```python
from build123d import *

# Parameters (mm, degrees)
BASE_PLATE_SKETCH_W        = 120
BASE_PLATE_SKETCH_H        = 72
BASE_PLATE_120X72X18_DEPTH = 9
CLAMP_RING_SKETCH_R        = 30
CLAMP_RING_SKETCH_R_2      = 24
CLAMP_RING_DEPTH           = 22
ARM_REACH                  = 190.308
ARM_END_RADIUS             = 30
ARM_PROFILE_SKETCH_W       = 26
ARM_PROFILE_SKETCH_H       = 48
CLAMP_LUG_DEPTH            = 13
CLAMP_LUG_EXTENSION_DEPTH  = 58
CLAMP_BOLT_HOLE_SKETCH_R   = 6
CLAMP_BOLT_HOLE_12_DEPTH   = 78
CLAMP_SPLIT_SLOT_SKETCH_W  = 44
CLAMP_SPLIT_SLOT_SKETCH_H  = 4
CLAMP_SPLIT_SLOT_4MM_DEPTH = 78
MOUNTING_SLOTS_2X_DEPTH    = 78


with BuildPart() as part:
    # Base Plate Sketch → Base Plate 120x72x18 (new, symmetric)
    with BuildSketch(Plane.XY):
        with Locations((60, 36)):
            Rectangle(BASE_PLATE_SKETCH_W, BASE_PLATE_SKETCH_H)
    extrude(amount=BASE_PLATE_120X72X18_DEPTH, both=True)



with BuildPart() as body_2:
    # Clamp Ring Sketch → Clamp Ring (new, symmetric)
    with BuildSketch(Plane(origin=(60, 0, 0), x_dir=(0, 0, -1), z_dir=(1, 0, 0))):
        with Locations(Location((-105, 36, 0), (0, 0, 180))):
            Circle(CLAMP_RING_SKETCH_R)
        with Locations(Location((-105, 36, 0), (0, 0, 180))):
            Circle(CLAMP_RING_SKETCH_R_2, mode=Mode.SUBTRACT)
    extrude(amount=CLAMP_RING_DEPTH, both=True)


with BuildPart() as part_1:
    add(part.part)

    add(body_2.part)  # Arm merges body 2
    # Arm: up to this cylinder (the profile starts outside it)
    arm_end = Plane(origin=(60, 36, 105), z_dir=(-1, 0, 0)) * Cylinder(ARM_END_RADIUS, 441.616, mode=Mode.PRIVATE)
    # Arm Profile Sketch → Arm (add, up to the surface)
    with BuildSketch(Plane.XY.offset(9), mode=Mode.PRIVATE) as arm_sk1:
        with Locations((60, 36)):
            Rectangle(ARM_PROFILE_SKETCH_W, ARM_PROFILE_SKETCH_H)
    arm_tool1 = extrude(arm_sk1.sketch, amount=ARM_REACH, mode=Mode.PRIVATE) - arm_end
    add(arm_tool1.solids().sort_by_distance((60, 36, 9))[0])

    # Clamp Lug Sketch → Clamp Lug (add, symmetric)
    with BuildSketch(Plane(origin=(60, 0, 0), x_dir=(0, 0, -1), z_dir=(1, 0, 0))):
        with BuildLine():
            Line((-153, 7), (-153, 65))
            Line((-153, 65), (-112.681145748, 65))
            ThreePointArc((-112.681145748, 65), (-135, 36), (-112.681145748, 7))
            Line((-112.681145748, 7), (-153, 7))
        make_face()
    extrude(amount=CLAMP_LUG_DEPTH, both=True)

    # Clamp Lug Extension Sketch → Clamp Lug Extension (add)
    with BuildSketch(Plane.XZ.offset(-7)):
        with BuildLine():
            Line((47, 153), (73, 153))
            ThreePointArc((73, 153), (60, 166), (47, 153))
        make_face()
    extrude(amount=-CLAMP_LUG_EXTENSION_DEPTH)

    # Clamp Bolt Hole Sketch → Clamp Bolt Hole Ø12 (cut)
    with BuildSketch(Plane.XZ.offset(-7)):
        with Locations(Location((60, 153, 0), (0, 0, 270))):
            Circle(CLAMP_BOLT_HOLE_SKETCH_R)
    extrude(amount=-CLAMP_BOLT_HOLE_12_DEPTH, mode=Mode.SUBTRACT)

    # Clamp Split Slot Sketch → Clamp Split Slot 4mm (cut)
    with BuildSketch(Plane.XY.offset(166)):
        with Locations((60, 35.211886187)):
            Rectangle(CLAMP_SPLIT_SLOT_SKETCH_W, CLAMP_SPLIT_SLOT_SKETCH_H)
    extrude(amount=-CLAMP_SPLIT_SLOT_4MM_DEPTH, mode=Mode.SUBTRACT)

    # Mounting Slots Sketch → Mounting Slots 2x (cut)
    with BuildSketch(Plane.XY.offset(9)):
        with BuildLine():
            Line((20.132428188, 47), (20.132428188, 25))
            ThreePointArc((20.132428188, 25), (14.132428188, 19), (8.132428188, 25))
            Line((8.132428188, 25), (8.132428188, 47))
            ThreePointArc((8.132428188, 47), (14.132428188, 53), (20.132428188, 47))
        make_face()
        with BuildLine():
            Line((99.867571812, 47), (99.867571812, 25))
            ThreePointArc((99.867571812, 25), (105.867571812, 19), (111.867571812, 25))
            Line((111.867571812, 25), (111.867571812, 47))
            ThreePointArc((111.867571812, 47), (105.867571812, 53), (99.867571812, 47))
        make_face()
    extrude(amount=-MOUNTING_SLOTS_2X_DEPTH, mode=Mode.SUBTRACT)


solid = part_1.part
```
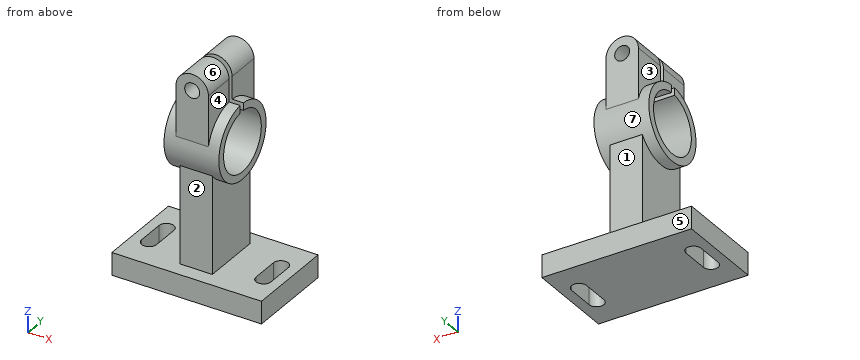
Geometry check sheet. Reference: the model listing, model coordinates, mm. Face numbers are marked on the shaded views. A direction names the side the tool comes from. Give positions to 0.01 mm unless a question says otherwise; leave off trailing zeros. Write each loop counter-clockwise with the first axis right and the second up, starting at its lowest first coordinate (ties: lowest second). Pieces come first, ordered by that corner, then holes.
1) Section check D-D, the plane y = 42.5. State how many separate pieces and enclosed holes the cut face has, and give its area (3 significant figures).
2) Release check for a two-part mould opening along Z. For the marked faces 5, 6 and 7 record: pulls with the +Z half, pulls with the -Z half, needs draft (parallel to the pull), parting line crosses it, or undercut.
3) Section check A-A, the plane z = 105. Record the boundary of the cut face in (x, y).
4) Access from +Z, -Z, +X, -X, +Y, -Y to the whole of each face (thin tool, end or side, straight path). Record for the marked faces 1, 2, 3 and 4.
5) Gauge pin test, flat ends, axial feed: pin 1 (8 mm diameter, centred on y = 24, z = 137.5, fed in from +X); pin 2 (13 mm diameter, centred on x = 64, z = 126.5, fed in from -Y); pin 3 (21 mm diameter, centred on x = 63, z = 148.5, fed in from +Y). Record the tip position at first contact, or that the pin passes through.
6) Section check C-C, the plane x = 16.5. Record the boundary of the cut face in (y, z).
7) Section check B-B, the plane y = 14. Record the boundary of the cut face in (x, z).
8) Material ranges on L1, parallel to X at y = 27.5, z = 3; L2, parallel to X at y = 19.5, z = 153; L3, parallel to Z at x = 74, y = 48.5, recorded low to high.
Computed:
1. separate pieces: 4
1. enclosed holes: 1
1. area: 4,650 mm2
2. face 5: needs draft
2. face 6: pulls with the +Z half
2. face 7: undercut
3. outline: (38, 6) - (82, 6) - (82, 12) - (38, 12) - close; (38, 60) - (82, 60) - (82, 66) - (38, 66) - close
4. face 1: +X, -X, +Y
4. face 2: +X, -X, -Y
4. face 3: +Z, -X, +Y
4. face 4: +Z, +X, -Y
5. pin 1: stops at x = 73
5. pin 2: stops at y = 7
5. pin 3: stops at y = 65
6. outline: (0, -9) - (19.49, -9) - (19.49, 9) - (0, 9) - close; (52.51, -9) - (72, -9) - (72, 9) - (52.51, 9) - close
7. outline: (0, -9) - (120, -9) - (120, 9) - (73, 9) - (73, 84.6) - (82, 84.6) - (82, 95.41) - (38, 95.41) - (38, 84.6) - (47, 84.6) - (47, 9) - (0, 9) - close; (38, 114.59) - (82, 114.59) - (82, 125.4) - (73, 125.4) - (73, 153) arc R13 ccw to (47, 153) - (47, 125.4) - (38, 125.4) - close; hole circle Ø12 at (60, 153)
8. L1: x = 0 to 8.13, 20.13 to 99.87, 111.87 to 120
8. L2: x = 47 to 54, 66 to 73
8. L3: z = -9 to 9, 77.73 to 84.51, 125.49 to 132.27
